Geometry check sheet. Reference: the model listing, model coordinates, mm. A direction names the side the tool comes from. Coordinates: 2 decimals unless noted, no trailing zeros. Write each loop counter-clockwise with the first axis right and the second up, starting at its lowest first coordinate (ties: lowest second). Pieces come first, ordered by that corner, then holes. Notation, with made-up numbers: (-9.5, -22) -> (21.5, -22) arc R19 ccw to (21.5, -2) -> close; hole circle Ø10 at (10, 60). An arc over 180 degrees is marked (long way). Answer in a Markdown table with one row per item. Add a question column.
1. Cross-section at B-B on x = 33. Record the cut outline in (y, z), and give its area (3 significant figures).
2. Scan lines: L1, parallel to Y at x = 0, z = 3.5; L2, parallel to Y at x = 0, z = 44; L3, parallel to X at y = 17, z = 10. Record each from-to range of solid material in increasing order. Write a range as from..to.
3. Set-up check for faces 4 (the cylindrical face through (-23.846, -7.509, 44.58)), 5 (the cylindrical face through (3, 39, 7)), 6 (the flat face through (-21.564, -31.432, 82.395)), 7 (the cylindrical face through (-13.887, -10.648, 74.79)), 8 (the cylindrical face through (-30, 0, 82)): record each of +Z, -Z, +X, -X, +Y, -Y from which the full face is reachable in a straight line by a thin tool's end or side.
4. Cross-section at A-A on y = 0. Record the cut outline in (x, z), and give its area (3 significant figures).
5. Depth check by flat-ended pin: P1, Ø8, axis at x = 33.5, y = -31, coming from the +Z side; P2, Ø1, axis at x = -11, z = 35, coming from the +Y side; P3, Ø11.5, axis at x = -30.31, y = 17.5, coming from the -Z side; P4, Ø1, axis at x = -8, z = 57, coming from the -Y side. Enter the tip coordinate at first touch or a pass-through.
6. Mould release check, pull along Z, two halves, no side actions. Record for faces 1 (the cylindrical face through (29.23, -22.38, 7.4)), 2 (the flat face through (10, -10, 0)), 3 (the flat face through (-11.6, 22.5, 15)): pulls with the +Z half, pulls with the -Z half, needs draft (parallel to the pull), parting line crosses it, or undercut.
7. Cross-section at D-D on z = 70.5. Record the cut outline in (x, y).
8. Cross-section at C-C on x = -10.5. Record the cut outline in (y, z).
```python
from build123d import *

# Parameters (mm, degrees)
ROUND_FLANGE_SKETCH_R       = 49
ROUND_FLANGE_SKETCH_R_2     = 13
ROUND_FLANGE_SKETCH_R_3     = 5
ROUND_FLANGE_98_6X_10_DEPTH = 15
TUBE_SKETCH_R               = 25
TUBE_SKETCH_R_2             = 13
TUBE_50_BORE_26_DEPTH       = 45
COLLAR_SKETCH_R             = 25
COLLAR_SKETCH_R_2           = 17.5
COLLAR_DEPTH                = 15
OVAL_FLANGE_SKETCH_R        = 25
OVAL_FLANGE_SKETCH_R_2      = 17.5
OVAL_FLANGE_SKETCH_R_3      = 15
OVAL_FLANGE_SKETCH_R_4      = 6
OVAL_FLANGE_2X_12_DEPTH     = 15


with BuildPart() as part:
    # Round Flange Sketch → Round Flange Ø98 6xØ10 (new body)
    with BuildSketch(Plane.XY):
        Circle(ROUND_FLANGE_SKETCH_R)
        Circle(ROUND_FLANGE_SKETCH_R_2, mode=Mode.SUBTRACT)
        with Locations((0, 35)):
            Circle(ROUND_FLANGE_SKETCH_R_3, mode=Mode.SUBTRACT)
        with Locations((30.310889132, 17.5)):
            Circle(ROUND_FLANGE_SKETCH_R_3, mode=Mode.SUBTRACT)
        with Locations((30.310889132, -17.5)):
            Circle(ROUND_FLANGE_SKETCH_R_3, mode=Mode.SUBTRACT)
        with Locations((0, -35)):
            Circle(ROUND_FLANGE_SKETCH_R_3, mode=Mode.SUBTRACT)
        with Locations((-30.310889132, -17.5)):
            Circle(ROUND_FLANGE_SKETCH_R_3, mode=Mode.SUBTRACT)
        with Locations((-30.310889132, 17.5)):
            Circle(ROUND_FLANGE_SKETCH_R_3, mode=Mode.SUBTRACT)
    extrude(amount=ROUND_FLANGE_98_6X_10_DEPTH)

    # Tube Sketch → Tube Ø50 Bore Ø26 (add)
    with BuildSketch(Plane.XY.offset(15)):
        with Locations(Location((0, 0, 0), (0, 0, 180))):
            Circle(TUBE_SKETCH_R)
        Circle(TUBE_SKETCH_R_2, mode=Mode.SUBTRACT)
    extrude(amount=TUBE_50_BORE_26_DEPTH)

    # Collar Sketch → Collar (add)
    with BuildSketch(Plane.XY.offset(60)):
        with Locations(Location((0, 0, 0), (0, 0, 180))):
            Circle(COLLAR_SKETCH_R)
        Circle(COLLAR_SKETCH_R_2, mode=Mode.SUBTRACT)
    extrude(amount=COLLAR_DEPTH)

    # Oval Flange Sketch → Oval Flange 2xØ12 (add)
    # profile 1 of 4: a face of its own
    with BuildSketch(Plane.XY.offset(75)):
        with BuildLine():
            Line((-14.309088021, 54.5), (-28.618176043, 9))
            ThreePointArc((-28.618176043, 9), (-30, 0), (-28.618176043, -9))
            Line((-28.618176043, -9), (-14.309088021, -54.5))
            ThreePointArc((-14.309088021, -54.5), (-2.276365489, -35.173734113), (15, -50))
            ThreePointArc((15, -50), (14.826265887, -52.276365489), (14.309088021, -54.5))
            Line((14.309088021, -54.5), (28.618176043, -9))
            ThreePointArc((28.618176043, -9), (30, 0), (28.618176043, 9))
            Line((28.618176043, 9), (14.309088021, 54.5))
            ThreePointArc((14.309088021, 54.5), (14.826265887, 52.276365489), (15, 50))
            ThreePointArc((15, 50), (-2.276365489, 35.173734113), (-14.309088021, 54.5))
        make_face()
        with Locations(Location((0, 0, 0), (0, 0, 180))):
            Circle(OVAL_FLANGE_SKETCH_R, mode=Mode.SUBTRACT)
    # profile 2 of 4: a face of its own
    with BuildSketch(Plane.XY.offset(75)):
        with Locations(Location((0, 0, 0), (0, 0, 180))):
            Circle(OVAL_FLANGE_SKETCH_R)
        Circle(OVAL_FLANGE_SKETCH_R_2, mode=Mode.SUBTRACT)
    # profile 3 of 4: a face of its own
    with BuildSketch(Plane.XY.offset(75)):
        with Locations((0, 50)):
            Circle(OVAL_FLANGE_SKETCH_R_3)
        with Locations((0, 50)):
            Circle(OVAL_FLANGE_SKETCH_R_4, mode=Mode.SUBTRACT)
    # profile 4 of 4: a face of its own
    with BuildSketch(Plane.XY.offset(75)):
        with Locations((0, -50)):
            Circle(OVAL_FLANGE_SKETCH_R_3)
        with Locations((0, -50)):
            Circle(OVAL_FLANGE_SKETCH_R_4, mode=Mode.SUBTRACT)
    extrude(amount=OVAL_FLANGE_2X_12_DEPTH)


solid = part.part
```
Results found:
| question | item | result |
|---|---|---|
| 1 | outline | (-36.22, 0) -> (-21.72, 0) -> (-21.72, 15) -> (-36.22, 15) -> close; (-13.28, 0) -> (13.28, 0) -> (13.28, 15) -> (-13.28, 15) -> close; (21.72, 0) -> (36.22, 0) -> (36.22, 15) -> (21.72, 15) -> close |
| 1 | area | 834 mm^2 |
| 2 | L1 | y = -49..-40, -30..-13, 13..30, 40..49 |
| 2 | L2 | y = -25..-13, 13..25 |
| 2 | L3 | x = -45.96..-35.29, -25.34..25.34, 35.29..45.96 |
| 3 | face 4 | none |
| 3 | face 5 | -Z |
| 3 | face 6 | +Z, -X, -Y |
| 3 | face 7 | +Z |
| 3 | face 8 | +Z, -X |
| 4 | outline | (-49, 0) -> (-13, 0) -> (-13, 60) -> (-17.5, 60) -> (-17.5, 90) -> (-30, 90) -> (-30, 75) -> (-25, 75) -> (-25, 15) -> (-49, 15) -> close; (13, 0) -> (49, 0) -> (49, 15) -> (25, 15) -> (25, 75) -> (30, 75) -> (30, 90) -> (17.5, 90) -> (17.5, 60) -> (13, 60) -> close |
| 4 | area | 2,760 mm^2 |
| 5 | P1 | stops at z = 15 |
| 5 | P2 | stops at y = 22.69 |
| 5 | P3 | stops at z = 0 |
| 5 | P4 | stops at y = -23.85 |
| 6 | face 1 | needs draft |
| 6 | face 2 | pulls with the -Z half |
| 6 | face 3 | undercut |
| 7 | outline | circle Ø50 at (0, 0); hole circle Ø35 at (0, 0) |
| 8 | outline | (-60.71, 75) -> (-22.69, 75) -> (-22.69, 15) -> (-47.86, 15) -> (-47.86, 0) -> (-7.66, 0) -> (-7.66, 60) -> (-14, 60) -> (-14, 90) -> (-60.71, 90) -> close; (7.66, 0) -> (47.86, 0) -> (47.86, 15) -> (22.69, 15) -> (22.69, 75) -> (60.71, 75) -> (60.71, 90) -> (14, 90) -> (14, 60) -> (7.66, 60) -> close |
